```python
from build123d import *

# Parameters (mm, degrees)
BASE_PLATE_SKETCH_W       = 120
BASE_PLATE_SKETCH_H       = 68
BASE_PLATE_DEPTH          = 25
HUB_SKETCH_R              = 17
HUB_34_DEPTH              = 48
LUG_DEPTH                 = 5
HUB_BORE_SKETCH_R         = 15
HUB_BORE_30_DEPTH         = 33
THROUGH_HOLE_SKETCH_R     = 9
THROUGH_HOLE_18_DEPTH     = 10
BOTTOM_BORE_SKETCH_R      = 15
BOTTOM_BORE_30_DEPTH      = 95.519839187
LUG_HOLE_SKETCH_R         = 5
LUG_HOLE_10_DEPTH         = 25
MOUNTING_SLOTS_2X20_DEPTH = 20
SLOT_RELIEF_SKETCH_R      = 4
SLOT_RELIEF_CUTS_DEPTH    = 20


with BuildPart() as part:
    # Base Plate Sketch → Base Plate (new body)
    with BuildSketch(Plane(origin=(0, 0, 0), x_dir=(1, 0, 0), z_dir=(0, 1, 0))):
        Rectangle(BASE_PLATE_SKETCH_W, BASE_PLATE_SKETCH_H)
    extrude(amount=BASE_PLATE_DEPTH)

    # Hub Sketch → Hub Ø34 (add)
    with BuildSketch(Plane(origin=(0, 25, 0), x_dir=(1, 0, 0), z_dir=(0, 1, 0))):
        with Locations(Location((-33, 0, 0), (0, 0, 90))):
            Circle(HUB_SKETCH_R)
    extrude(amount=HUB_34_DEPTH)

    # Lug Sketch → Lug (add, symmetric)
    with BuildSketch(Plane.XY):
        with BuildLine():
            Line((-65, 68), (-48.898372545, 68))
            Line((-48.898372545, 68), (-48.898372545, 44))
            Line((-48.898372545, 44), (-65, 44))
            ThreePointArc((-65, 44), (-77, 56), (-65, 68))
        make_face()
    extrude(amount=LUG_DEPTH, both=True)

    # Hub Bore Sketch → Hub Bore Ø30 (cut)
    with BuildSketch(Plane(origin=(0, 73, 0), x_dir=(1, 0, 0), z_dir=(0, 1, 0))):
        with Locations(Location((-33, 0, 0), (0, 0, 270))):
            Circle(HUB_BORE_SKETCH_R)
    extrude(amount=-HUB_BORE_30_DEPTH, mode=Mode.SUBTRACT)

    # Through Hole Sketch → Through Hole Ø18 (cut)
    with BuildSketch(Plane(origin=(0, 40, 0), x_dir=(1, 0, 0), z_dir=(0, 1, 0))):
        with Locations(Location((-33, 0, 0), (0, 0, 270))):
            Circle(THROUGH_HOLE_SKETCH_R)
    extrude(amount=-THROUGH_HOLE_18_DEPTH, mode=Mode.SUBTRACT)

    # Bottom Bore Sketch → Bottom Bore Ø30 (cut, through all)
    with BuildSketch(Plane(origin=(0, 30, 0), x_dir=(1, 0, 0), z_dir=(0, 1, 0))):
        with Locations(Location((-33, 0, 0), (0, 0, 270))):
            Circle(BOTTOM_BORE_SKETCH_R)
    extrude(amount=-BOTTOM_BORE_30_DEPTH, mode=Mode.SUBTRACT)

    # Lug Hole Sketch → Lug Hole Ø10 (cut)
    with BuildSketch(Plane.XY.offset(5)):
        with Locations((-65, 56)):
            Circle(LUG_HOLE_SKETCH_R)
    extrude(amount=-LUG_HOLE_10_DEPTH, mode=Mode.SUBTRACT)

    # Mounting Slots Sketch → Mounting Slots 2x20 (cut)
    with BuildSketch(Plane(origin=(0, 25, 0), x_dir=(1, 0, 0), z_dir=(0, 1, 0))):
        with BuildLine():
            Line((42, 27), (60, 27))
            Line((60, 27), (60, 7))
            Line((60, 7), (42, 7))
            ThreePointArc((42, 7), (32, 17), (42, 27))
        make_face()
        with BuildLine():
            Line((42, -7), (60, -7))
            Line((60, -7), (60, -27))
            Line((60, -27), (42, -27))
            ThreePointArc((42, -27), (32, -17), (42, -7))
        make_face()
    extrude(amount=-MOUNTING_SLOTS_2X20_DEPTH, mode=Mode.SUBTRACT)

    # Slot Relief Sketch → Slot Relief Cuts (cut)
    with BuildSketch(Plane(origin=(0, 5, 0), x_dir=(1, 0, 0), z_dir=(0, 1, 0))):
        with Locations(Location((42, 17, 0), (0, 0, 270))):
            Circle(SLOT_RELIEF_SKETCH_R)
        with Locations(Location((42, -17, 0), (0, 0, 270))):
            Circle(SLOT_RELIEF_SKETCH_R)
    extrude(amount=-SLOT_RELIEF_CUTS_DEPTH, mode=Mode.SUBTRACT)


solid = part.part
```
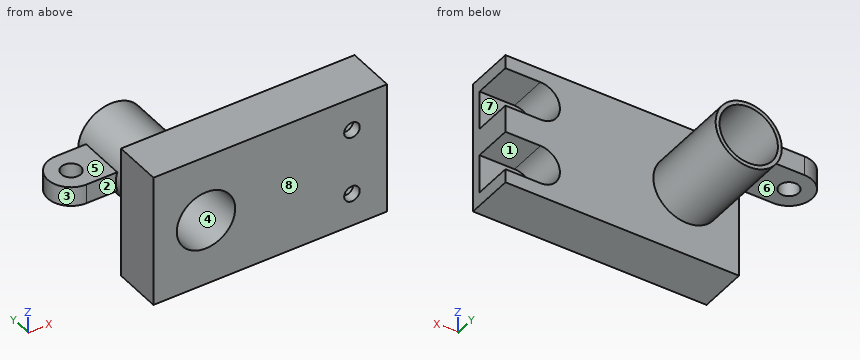
The listing builds one solid part. Answer for the finished solid, in the listing's coordinates (mm). Face numbers are marked on the shaded views. A direction names the side the tool comes from. Round coordinates to 2 decimals unless told otherwise and drop trailing zeros. Write each loop counter-clockwise with the first axis right and the second up, starting at its lowest first coordinate (ties: lowest second). Pieces come first, ordered by that corner, then holes. Notation, with made-up numbers: (70, 1) -> (106, 1) arc R30 cw to (106, 39) -> close; hole circle Ø3 at (80.5, -34). An arc over 180 degrees is marked (long way). Write item = value, one per line.
1) Straight lines are drawn through the part: line 1 along Z through (x, y) = (40, 19.5); line 2 along X through (y, z) = (1, 17); line 3 along Y through (x, z) = (5.5, -21). For each, find the intervals that lie inside material, in ascending order. Write a range as [from, to].
Check values:
line_1 = [-34, -26.8], [-7.2, 7.2], [26.8, 34]
line_2 = [-60, 38], [46, 60]
line_3 = [0, 25]
2) Given pin 1 (19 mm diameter, centred on x = -61.5, y = 59.5, fed in from +Z); pin 2 (5 mm diameter, centred on x = -37, z = 22, fed in from +Y); pin 3 (9 mm diameter, centred on x = -40, z = 1, fed in from +Y); pin 4 (9 mm diameter, centred on x = -65, y = 56, fed in from +Z), each flat-ended and moving along its own axis, determine where each tip first touches the part or whether it passes through.
Check values:
pin_1 = 5
pin_2 = 25
pin_3 = 40
pin_4 = through
3) Section B-B on y = 56 is taken. Write down the section's boundary in (x, z).
Check values:
outline = (-77, -5) -> (-70, -5) -> (-70, 5) -> (-77, 5) -> close; (-60, -5) -> (-49.25, -5) arc R17 ccw (long way) to (-49.25, 5) -> (-60, 5) -> close; hole circle Ø30 at (-33, 0)
4) Section A-A on z = 0 is taken. Write down the section's boundary in (x, y), plus the area to 3 significant figures.
Check values:
outline = (-65, 44) -> (-50, 44) -> (-50, 25) -> (-60, 25) -> (-60, 0) -> (-48, 0) -> (-48, 30) -> (-42, 30) -> (-42, 40) -> (-48, 40) -> (-48, 73) -> (-50, 73) -> (-50, 68) -> (-65, 68) arc R12 ccw to start; (-24, 30) -> (-18, 30) -> (-18, 0) -> (60, 0) -> (60, 25) -> (-16, 25) -> (-16, 73) -> (-18, 73) -> (-18, 40) -> (-24, 40) -> close; hole circle Ø10 at (-65, 56)
area = 3,070 mm²
5) For a pull along Y with two mould halves and no side action, classify the marked faces 1, 2 and 3 as released by +Y, released by -Y, zero draft, split by the parting line, or undercut.
Check values:
face_1 = zero draft
face_2 = undercut
face_3 = split by the parting line
6) Section C-C on x = -67 is taken. Write down the section's boundary in (y, z), plus the area to 3 significant figures.
Check values:
outline = (44.17, -5) -> (51.42, -5) -> (51.42, 5) -> (44.17, 5) -> close; (60.58, -5) -> (67.83, -5) -> (67.83, 5) -> (60.58, 5) -> close
area = 145 mm²
7) Which of the six approach directions +Z, -Z, +X, -X, +Y, -Y give full straight-line access (tool end or side, diameter ignored) to the marked faces 4, 5, 6, 7 and 8?
Check values:
face_4 = -Y
face_5 = +Z, -X, +Y
face_6 = -Z, -X, +Y
face_7 = +X, +Y
face_8 = +Z, -Z, +X, -X, -Y
8) Section D-D on y = 12 is taken. Write down the section's boundary in (x, z).
Check values:
outline = (-60, -34) -> (60, -34) -> (60, -27) -> (42, -27) arc R10 cw to (42, -7) -> (60, -7) -> (60, 7) -> (42, 7) arc R10 cw to (42, 27) -> (60, 27) -> (60, 34) -> (-60, 34) -> close; hole circle Ø30 at (-33, 0)
